Geometry: final body of the model. Coordinates: model frame, mm. Round coordinates to 2 decimals unless told otherwise and drop trailing zeros. Loops run counter-clockwise (first coordinate to the right, second up) from the corner with the lowest first, then second, coordinate; pieces in that order, holes last. Notation, with made-up numbers: (62, 51.5) - (93, 51.5) arc R21 ccw to (93, 84.5) - close; hole circle Ø6 at (14.5, 41). An arc over 180 degrees is marked (long way). Return JSON: item names as keys, results as strings. Group by question number.
1. Section B-B on y = 0. Return loops of the section in (x, z), and give its area (3 significant figures).
2. Draft query along Y for faces 1 (the face through (0, -8, 0)), 2 (the face through (25, 0, 0)), 3 (the face through (-10.976, -0.632, 0.038)), 4 (the face through (0, 8, 0)). Return one class per face: +Y half, -Y half, draft (parallel to the pull), parting line (faces both ways), or undercut.
3. Section C-C on z = 0.9. Return loops of the section in (x, y), and give its area (3 significant figures).
4. First-contact query: pin 1 Ø4.5 at (x, y) = (-12.5, 0) entering from -Z; pin 2 Ø2.5 at (x, y) = (12.5, 0) entering from +Z. Flat tips, straight axial feed; report the tip coordinate or a pass-through.
5. Material intervals for probe 1 along Y at (x, z) = (-12.5, 0.65); probe 2 along Y at (x, z) = (-11.5, -2.15); probe 3 along X at (y, z) = (-7.5, 0.55), sorted ascending.
6. Section A-A on x = 12.5. Return loops of the section in (y, z), and give its area (4 significant figures).
from build123d import *

# Parameters (mm, degrees)
SKETCH_1_W         = 50
SKETCH_1_H         = 16
EXTRUDE_1_DEPTH    = 2.75
HOLE_WIZARD_M4_1_D = 3.3
CHAMFER_1_SIZE     = 1


with BuildPart() as part:
    # 草图1 → 凸台-拉伸1 (new, symmetric)
    with BuildSketch(Plane.XY):
        Rectangle(SKETCH_1_W, SKETCH_1_H)
    extrude(amount=EXTRUDE_1_DEPTH, both=True)

    # M4 螺纹孔1 (through all)
    with Locations(Plane(origin=(0, 0, -2.75), x_dir=(-1, 0, 0), z_dir=(0, 0, -1))):
        with Locations((12.5, 0), (-12.5, 0)):
            Hole(HOLE_WIZARD_M4_1_D / 2)

    # 倒角1
    chamfer_1_edges = [part.edges().sort_by_distance(p)[0] for p in [
        (25, -8, 0),
        (-25, -8, 0),
        (-25, 8, 0),
        (25, 8, 0),
    ]]
    chamfer(chamfer_1_edges, length=CHAMFER_1_SIZE)


solid = part.part
Taken from the geometry:
{
 "1": {"outline": "(-25, -2.75) - (-14.15, -2.75) - (-14.15, 2.75) - (-25, 2.75) - close; (-10.85, -2.75) - (10.85, -2.75) - (10.85, 2.75) - (-10.85, 2.75) - close; (14.15, -2.75) - (25, -2.75) - (25, 2.75) - (14.15, 2.75) - close", "area": "239 mm2"},
 "2": {"face 1": "-Y half", "face 2": "draft", "face 3": "undercut", "face 4": "+Y half"},
 "3": {"outline": "(-25, -7) - (-24, -8) - (24, -8) - (25, -7) - (25, 7) - (24, 8) - (-24, 8) - (-25, 7) - close; hole circle Ø3.3 at (-12.5, 0); hole circle Ø3.3 at (12.5, 0)", "area": "781 mm2"},
 "4": {"pin 1": "z = -2.75", "pin 2": "through"},
 "5": {"probe 1": "-8 to -1.65, 1.65 to 8", "probe 2": "-8 to -1.31, 1.31 to 8", "probe 3": "-24.5 to 24.5"},
 "6": {"outline": "(-8, -2.75) - (-1.65, -2.75) - (-1.65, 2.75) - (-8, 2.75) - close; (1.65, -2.75) - (8, -2.75) - (8, 2.75) - (1.65, 2.75) - close", "area": "69.85 mm2"}
}
